Check sheet for the drawn part. Datum: minimum x, y, z corner. Units: mm. A direction names the side the tool comes from. Give positions to 0.01 mm unless a question says otherwise; leave off trailing zeros. Order: outer loops, then holes, each group sorted by start corner. A loop starts at its lowest first (then second) coordinate and runs counter-clockwise, first axis right, second up. Notation, with made-up numbers: M 49,42 L 67,42 A38 ccw 67,80 Z; hole C 73,77.25 d10. An arc over 180 degrees is marked long. Put each result on its own line as item: value. Start each with the question number.
Q1. Material ranges on L1, parallel to X at y = 1.75, z = 4.75; L2, parallel to X at y = 6, z = 2.25; L3, parallel to Z at x = 14.25, y = 1.5, recorded low to high.
Q2. Access from +Z, -Z, +X, -X, +Y, -Y to the whole of each face (thin tool, end or side, straight path). Record for the marked faces 1, 2 and 3.
Q3. Section check A-A on y = 3.5. Record the cut outline in (x, z).
Q4. Go/stop test with flat-tipped pins: pin 1 (3 mm diameter, centred on y = 2, z = 2, fed in from -X); pin 2 (1 mm diameter, centred on x = 18, y = 5.5, fed in from +Z). Record where each tip stops, or that it passes through.
Q5. Section check D-D on y = 5.5. Record the cut outline in (x, z), then the cut area to 3 significant figures.
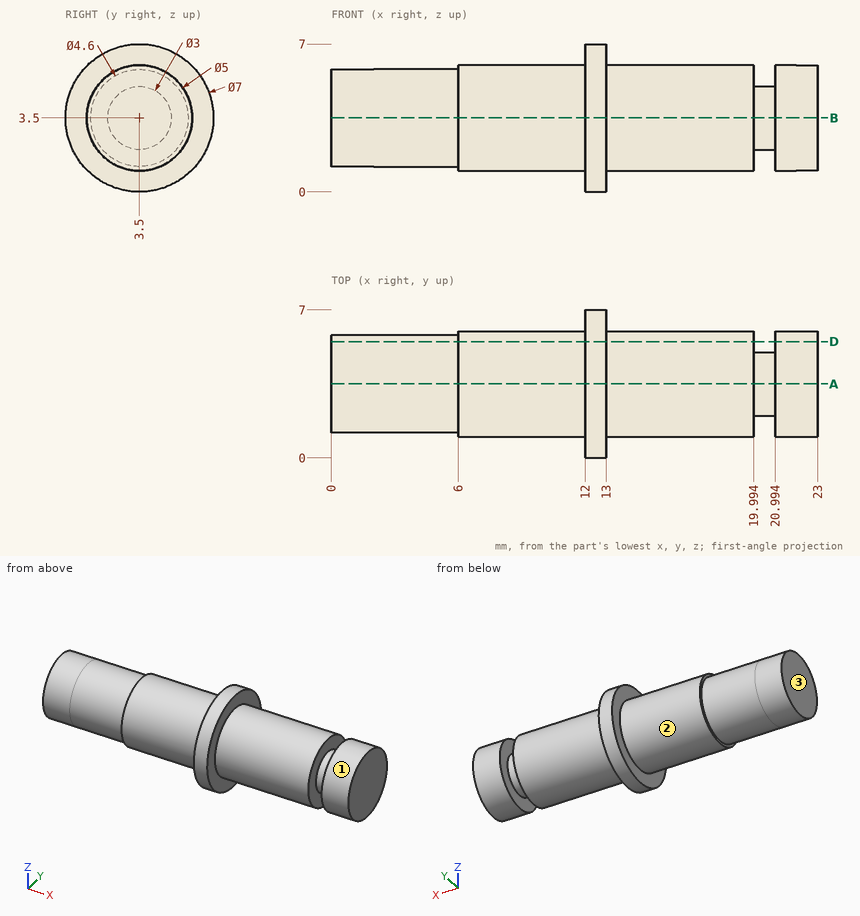
Results found:
1. L1: x = 0 to 19.99, 20.99 to 23
1. L2: x = 12 to 13
1. L3: z = 2 to 5
2. face 1: +X
2. face 2: -X
2. face 3: +Z, -Z, -X, +Y, -Y
3. outline: M 0,1.2 L 6,1.2 L 6,1 L 12,1 L 12,0 L 13,0 L 13,1 L 19.99,1 L 19.99,2 L 20.99,2 L 20.99,1 L 23,1 L 23,6 L 20.99,6 L 20.99,5 L 19.99,5 L 19.99,6 L 13,6 L 13,7 L 12,7 L 12,6 L 6,6 L 6,5.8 L 0,5.8 Z
4. pin 1: stops at x = 0
4. pin 2: stops at z = 5.5
5. outline: M 0,2.36 L 6,2.36 L 6,2 L 12,2 L 12,0.63 L 13,0.63 L 13,2 L 19.99,2 L 19.99,5 L 13,5 L 13,6.37 L 12,6.37 L 12,5 L 6,5 L 6,4.64 L 0,4.64 Z; M 20.99,2 L 23,2 L 23,5 L 20.99,5 Z
5. area: 64.4 mm^2
